```python
from build123d import *

# Parameters (mm, degrees)
SKETCH_1_W          = 263
SKETCH_1_H          = 243
EXTRUDE_1_DEPTH     = 3
SKETCH_4_R          = 2.2
CUT_EXTRUDE_2_DEPTH = 10
SKETCH_5_R          = 3.3
CUT_EXTRUDE_3_DEPTH = 10


with BuildPart() as part:
    # 草图1 → 凸台-拉伸1 (new body)
    with BuildSketch(Plane.XY):
        Rectangle(SKETCH_1_W, SKETCH_1_H)
    extrude(amount=EXTRUDE_1_DEPTH)

    # 草图4 → 切除-拉伸2 (cut)
    with BuildSketch(Plane(origin=(0, 0, 0), x_dir=(-1, 0, 0), z_dir=(0, 0, -1))):
        with Locations((-122.5, -68.5)):
            Circle(SKETCH_4_R)
        with Locations((-122.5, -93.5)):
            Circle(SKETCH_4_R)
    cut_extrude_2 = extrude(amount=-CUT_EXTRUDE_2_DEPTH, mode=Mode.SUBTRACT)

    # 镜向1: 切除-拉伸2 across plane
    add(cut_extrude_2.mirror(Plane.ZX), mode=Mode.SUBTRACT)

    # 草图5 → 切除-拉伸3 (cut)
    with BuildSketch(Plane.XY.offset(3)):
        with Locations((-95.5, 0)):
            Circle(SKETCH_5_R)
    extrude(amount=-CUT_EXTRUDE_3_DEPTH, mode=Mode.SUBTRACT)


solid = part.part
```
Input: part model. Units: mm. Frame: model coordinates. Round coordinates to 2 decimals unless told otherwise and drop trailing zeros. Loops run counter-clockwise (first coordinate to the right, second up) from the corner with the lowest first, then second, coordinate; pieces in that order, holes last. Notation, with made-up numbers: (40, 55) - (56, 55) arc R15 cw to (56, 77) - close; hole circle Ø3 at (38.5, -32). An arc over 180 degrees is marked (long way). One line per item, written item: value. Start each with the question number.
(1) Section A-A, the plane y = 0. Return loops of the section in (x, z), plus the area to 3 significant figures.
(2) Ray query, line 1 (X direction, y = 93.5, z = 1.2); line 2 (X direction, y = -1, z = 0.45); line 3 (Y direction, x = -98.5, z = 0.75). Return the intervals inside material, ascending. Write a range as [from, to].
(3) Section B-B, the plane x = -95.5. Return loops of the section in (y, z).
(4) Draft query along Y for faces 1 (the cylindrical face through (-98.8, 0.1, 1.5)), 2 (the flat face through (-2, 2, 3)). Return one class per face: +Y half, -Y half, draft (parallel to the pull), parting line (faces both ways), or undercut.
(5) Contact query for a flat-ended pin moving along its axis: P1, Ø5, axis at x = -73.5, y = 63.5, coming from the -Z side. Output: stop coordinate, or through.
Results below:
1. outline: (-131.5, 0) - (-98.8, 0) - (-98.8, 3) - (-131.5, 3) - close; (-92.2, 0) - (131.5, 0) - (131.5, 3) - (-92.2, 3) - close
1. area: 769 mm^2
2. line 1: [-131.5, 120.3], [124.7, 131.5]
2. line 2: [-131.5, -98.64], [-92.36, 131.5]
2. line 3: [-121.5, -1.37], [1.37, 121.5]
3. outline: (-121.5, 0) - (-3.3, 0) - (-3.3, 3) - (-121.5, 3) - close; (3.3, 0) - (121.5, 0) - (121.5, 3) - (3.3, 3) - close
4. face 1: undercut
4. face 2: draft
5. P1: z = 0
